from build123d import *

# Parameters (mm, degrees)
SKETCH1_W                                           = 300
SKETCH1_H                                           = 200
BOSS_EXTRUDE1_DEPTH                                 = 5
SKETCH2_R                                           = 7.5
CUT_EXTRUDE1_DEPTH                                  = 10
LPATTERN1_COUNT                                     = 2
LPATTERN1_PITCH                                     = 180
LPATTERN1_COUNT_DIR2                                = 3
LPATTERN1_PITCH_DIR2                                = 80
HOLE_SIZE_BASED_ON_SOCKET_HEAD_CAP_SCRE_D           = 6.6
HOLE_SIZE_BASED_ON_SOCKET_HEAD_CAP_SCRE_CBORE_D     = 11
HOLE_SIZE_BASED_ON_SOCKET_HEAD_CAP_SCRE_CBORE_DEPTH = 6.8
CUT_EXTRUDE2_DEPTH                                  = 10
CUT_EXTRUDE3_DEPTH                                  = 6.8


with BuildPart() as part:
    # Sketch1 → Boss-Extrude1 (new, symmetric)
    with BuildSketch(Plane(origin=(0, 0, 0), x_dir=(1, 0, 0), z_dir=(0, 1, 0))):
        Rectangle(SKETCH1_W, SKETCH1_H)
    extrude(amount=BOSS_EXTRUDE1_DEPTH, both=True)

    # Sketch2 → Cut-Extrude1 (cut)
    with BuildSketch(Plane(origin=(0, 5, 0), x_dir=(1, 0, 0), z_dir=(0, 1, 0))):
        with Locations(Location((80, 90, 0), (0, 0, 270))):
            Circle(SKETCH2_R)
    cut_extrude1 = extrude(amount=-CUT_EXTRUDE1_DEPTH, mode=Mode.SUBTRACT)

    # LPattern1: Cut-Extrude1 2 × 3
    with Locations(*[(-j * LPATTERN1_PITCH_DIR2, 0, i * LPATTERN1_PITCH) for i in range(LPATTERN1_COUNT) for j in range(LPATTERN1_COUNT_DIR2) if (i, j) != (0, 0)]):
        add(cut_extrude1, mode=Mode.SUBTRACT)

    # Hole Size (based on socket head cap screw type)1 (through all)
    with Locations(Plane(origin=(0, 5, 0), x_dir=(1, 0, 0), z_dir=(0, 1, 0))):
        with Locations((-80, 25), (-80, -25)):
            CounterBoreHole(HOLE_SIZE_BASED_ON_SOCKET_HEAD_CAP_SCRE_D / 2, HOLE_SIZE_BASED_ON_SOCKET_HEAD_CAP_SCRE_CBORE_D / 2, HOLE_SIZE_BASED_ON_SOCKET_HEAD_CAP_SCRE_CBORE_DEPTH)

    # Sketch6 → Cut-Extrude2 (cut)
    with BuildSketch(Plane(origin=(0, 5, 0), x_dir=(1, 0, 0), z_dir=(0, 1, 0))):
        with BuildLine():
            Line((125, 21.7), (95, 21.7))
            ThreePointArc((95, 21.7), (91.7, 25), (95, 28.3))
            Line((95, 28.3), (125, 28.3))
            ThreePointArc((125, 28.3), (128.3, 25), (125, 21.7))
        make_face()
        with BuildLine():
            Line((125, -28.3), (95, -28.3))
            ThreePointArc((95, -28.3), (91.7, -25), (95, -21.7))
            Line((95, -21.7), (125, -21.7))
            ThreePointArc((125, -21.7), (128.3, -25), (125, -28.3))
        make_face()
    extrude(amount=-CUT_EXTRUDE2_DEPTH, mode=Mode.SUBTRACT)

    # Sketch7 → Cut-Extrude3 (cut)
    with BuildSketch(Plane(origin=(0, 5, 0), x_dir=(1, 0, 0), z_dir=(0, 1, 0))):
        with BuildLine():
            Line((125, 19.5), (95, 19.5))
            ThreePointArc((95, 19.5), (89.5, 25), (95, 30.5))
            Line((95, 30.5), (125, 30.5))
            ThreePointArc((125, 30.5), (130.5, 25), (125, 19.5))
        make_face()
        with BuildLine():
            Line((125, -30.5), (95, -30.5))
            ThreePointArc((95, -30.5), (89.5, -25), (95, -19.5))
            Line((95, -19.5), (125, -19.5))
            ThreePointArc((125, -19.5), (130.5, -25), (125, -30.5))
        make_face()
    extrude(amount=-CUT_EXTRUDE3_DEPTH, mode=Mode.SUBTRACT)


solid = part.part
Could you check a few things on this model? Use its own coordinates, in mm. A direction names the side the tool comes from. Give positions to 0.01 mm unless a question says otherwise; leave off trailing zeros. Write each loop counter-clockwise with the first axis right and the second up, starting at its lowest first coordinate (ties: lowest second). Pieces come first, ordered by that corner, then holes. Notation, with made-up numbers: (83, 31) -> (99, 31) arc R36 cw to (99, 67) -> close; hole circle Ø2 at (-16.5, 74.25). An arc over 180 degrees is marked (long way). Answer as a JSON object with one key per item and string values.
Q1. Suppose I cut it at C-C on x = 80. Write out the boundary of the cut face in (y, z).
Taken from the geometry:
{"outline": "(-5, -100) -> (5, -100) -> (5, -97.5) -> (-5, -97.5) -> close; (-5, -82.5) -> (5, -82.5) -> (5, 82.5) -> (-5, 82.5) -> close; (-5, 97.5) -> (5, 97.5) -> (5, 100) -> (-5, 100) -> close"}
Q2. We'd pull the mould along X, two halves only. Please class faces 3 (the flat face through (150, 0, 1)), 4 (the flat face through (110, -1.8, -21)), 5 (the flat face through (-2, -5, -1)), 6 (the cylindrical face through (5.1, 0.1, -95.5)): released by +X, released by -X, zero draft, split by the parting line, or undercut.
Taken from the geometry:
{"face 3": "released by +X", "face 4": "undercut", "face 5": "zero draft", "face 6": "undercut"}
Q3. Suppose I cut it at A-A on x = -80. Write out the boundary of the cut face in (y, z).
Taken from the geometry:
{"outline": "(-5, -100) -> (5, -100) -> (5, -97.5) -> (-5, -97.5) -> close; (-5, -82.5) -> (5, -82.5) -> (5, -30.5) -> (-1.8, -30.5) -> (-1.8, -28.3) -> (-5, -28.3) -> close; (-5, -21.7) -> (-1.8, -21.7) -> (-1.8, -19.5) -> (5, -19.5) -> (5, 19.5) -> (-1.8, 19.5) -> (-1.8, 21.7) -> (-5, 21.7) -> close; (-5, 28.3) -> (-1.8, 28.3) -> (-1.8, 30.5) -> (5, 30.5) -> (5, 82.5) -> (-5, 82.5) -> close; (-5, 97.5) -> (5, 97.5) -> (5, 100) -> (-5, 100) -> close"}
Q4. Suppose I cut it at B-B on z = 90. Write out the boundary of the cut face in (x, y).
Taken from the geometry:
{"outline": "(-150, -5) -> (-87.5, -5) -> (-87.5, 5) -> (-150, 5) -> close; (-72.5, -5) -> (-7.5, -5) -> (-7.5, 5) -> (-72.5, 5) -> close; (7.5, -5) -> (72.5, -5) -> (72.5, 5) -> (7.5, 5) -> close; (87.5, -5) -> (150, -5) -> (150, 5) -> (87.5, 5) -> close"}
Q5. Please list where these lines run through material, in increasing order: L1, parallel to X at y = -3, z = 90; L2, parallel to X at y = 0, z = -25; L3, parallel to Z at x = 98.5, y = -0.25.
Taken from the geometry:
{"L1": "x = -150 to -87.5, -72.5 to -7.5, 7.5 to 72.5, 87.5 to 150", "L2": "x = -150 to -85.5, -74.5 to 89.5, 130.5 to 150", "L3": "z = -100 to -30.5, -19.5 to 19.5, 30.5 to 100"}
Q6. Which directions (+Z, -Z, +X, -X, +Y, -Y) give clear straight access to the entire face, cutting with the end or side of a thin tool? Please do faces 1 (the cylindrical face through (89.5, 1.6, 25.1)), 2 (the cylindrical face through (5.1, 0.1, 84.5)).
Taken from the geometry:
{"face 1": "+Y", "face 2": "+Y, -Y"}
Q7. Will these pins go through, and if not, where does the flat tip stop? pin 1 Ø13.5 at (x, z) = (0, 90) entering from -Y; pin 2 Ø10 at (x, z) = (-80, -25) entering from +Y.
Taken from the geometry:
{"pin 1": "passes through", "pin 2": "stops at y = -1.8"}
Q8. Suppose I cut it at D-D on y = 0.25. Count the separate pieces of the cut face and the enclosed holes in it, then the cut area to 3 significant figures.
Taken from the geometry:
{"separate pieces": "1", "enclosed holes": "10", "area": "57,900 mm²"}
